Print and shaded views of the part. All mm, measured from the part's lowest x, y and z. Round coordinates to 2 decimals unless told otherwise and drop trailing zeros. Order: outer loops, then holes, each group sorted by start corner. A loop starts at its lowest first (then second) coordinate and runs counter-clockwise, first axis right, second up. Notation, with made-up numbers: (81.25, 76.25) -> (140.25, 76.25) arc R16 ccw to (140.25, 93.25) -> close; hole circle Ø8 at (87, 43.5). An arc over 180 degrees is marked (long way). Answer as CSV lines item,"result". Start each with the question number.
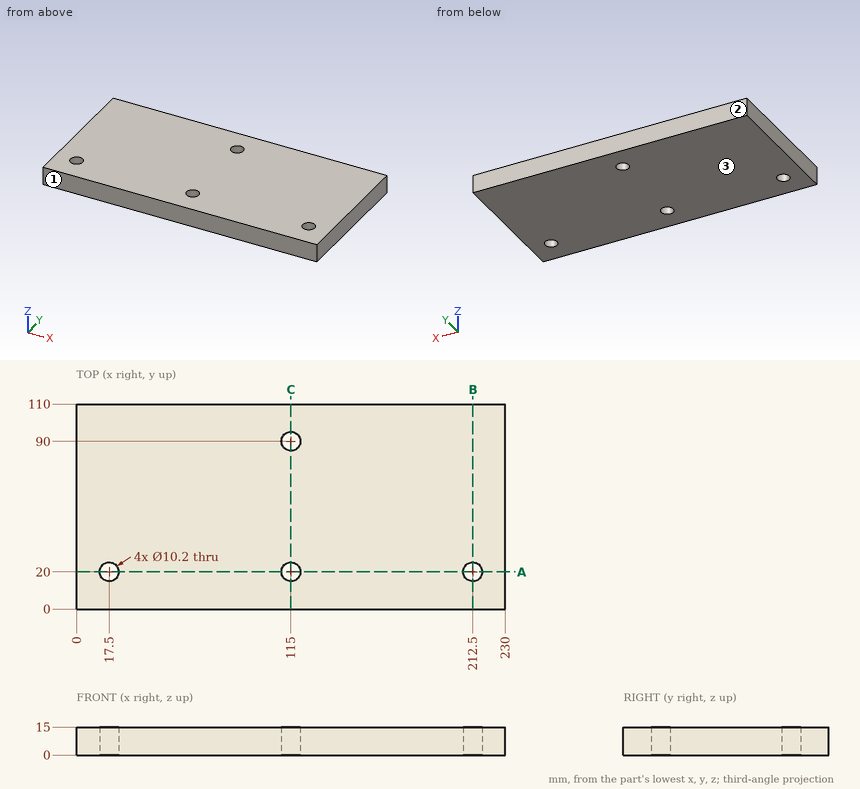
Item 1: Probe line 1 (Y direction, x = 115, z = 7.5); line 2 (Y direction, x = 17.5, z = 4.75); line 3 (X direction, y = 85.5, z = 10). List the from-to ranges inside material, lowest first.
Item 2: Band-saw the part on A-A, the plane y = 20. Give the cut face in (x, z).
Item 3: Band-saw the part on B-B, the plane x = 212.5. Give the cut face in (y, z), and give its area (3 significant figures).
Item 4: Pin check, flat tips, straight feed: pin 1 (4 mm diameter, centred on x = 43, y = 85.5, fed in from -Z); pin 2 (6 mm diameter, centred on x = 115, y = 20, fed in from +Z). Stop position of each tip, or through.
Item 5: Band-saw the part on C-C, the plane x = 115. Give the cut face in (y, z).
Item 6: Mould opens along Y. For the marked faces 1, 2 and 3 say: released by +Y, released by -Y, zero draft, split by the parting line, or undercut.
Values:
1,line 1,"0 to 14.9, 25.1 to 84.9, 95.1 to 110"
1,line 2,"0 to 14.9, 25.1 to 110"
1,line 3,"0 to 112.6, 117.4 to 230"
2,outline,"(0, 0) -> (12.4, 0) -> (12.4, 15) -> (0, 15) -> close; (22.6, 0) -> (109.9, 0) -> (109.9, 15) -> (22.6, 15) -> close; (120.1, 0) -> (207.4, 0) -> (207.4, 15) -> (120.1, 15) -> close; (217.6, 0) -> (230, 0) -> (230, 15) -> (217.6, 15) -> close"
3,outline,"(0, 0) -> (14.9, 0) -> (14.9, 15) -> (0, 15) -> close; (25.1, 0) -> (110, 0) -> (110, 15) -> (25.1, 15) -> close"
3,area,"1,500 mm²"
4,pin 1,"z = 0"
4,pin 2,"through"
5,outline,"(0, 0) -> (14.9, 0) -> (14.9, 15) -> (0, 15) -> close; (25.1, 0) -> (84.9, 0) -> (84.9, 15) -> (25.1, 15) -> close; (95.1, 0) -> (110, 0) -> (110, 15) -> (95.1, 15) -> close"
6,face 1,"released by -Y"
6,face 2,"released by +Y"
6,face 3,"zero draft"
